Could you check a few things on this drawing? It's one solid part, dimensions in mm from its lowest x, y, z. Coordinates: 2 decimals unless noted, no trailing zeros. Order: outer loops, then holes, each group sorted by start corner. A loop starts at its lowest first (then second) coordinate and runs counter-clockwise, first axis right, second up. Notation, with made-up numbers: (-15, 24.5) - (41, 24.5) arc R19 ccw to (41, 46.5) - close; hole circle Ø3 at (88.5, -37.5). An arc over 180 degrees is marked (long way). Return JSON: item names as keys, results as strings. Group by question number.
1) Imagine slicing it at A-A (z = 0.85). Write out the boundary of the cut face in (x, y), and give its area (3 significant figures).
2) Imagine slicing it at B-B (y = 17.5). Write out the boundary of the cut face in (x, z), and give its area (3 significant figures).
3) If I drill on line 1 along Y through (x, z) = (230, 1.5); line 2 along X through (y, z) = (9, 2.2); line 3 along X through (y, z) = (13, 0.8), over which ranges is the centre line in solid material (lowest first)?
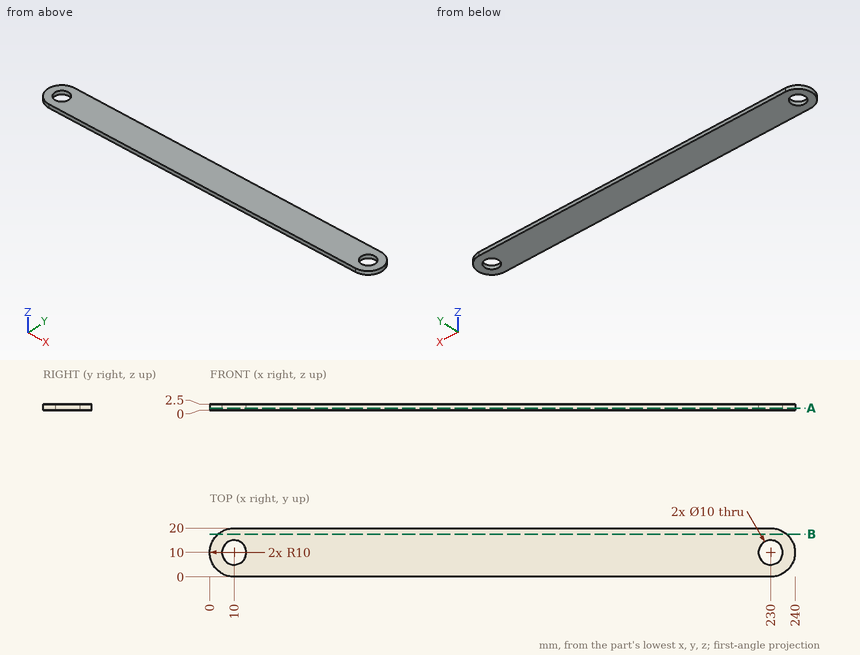
Calculated:
{
 "1": {"outline": "(10, 0) - (230, 0) arc R10 ccw to (230, 20) - (10, 20) arc R10 ccw to start; hole circle Ø10 at (10, 10); hole circle Ø10 at (230, 10)", "area": "4,560 mm2"},
 "2": {"outline": "(3.39, 0) - (236.61, 0) - (236.61, 2.5) - (3.39, 2.5) - close", "area": "583 mm2"},
 "3": {"line 1": "0 to 5, 15 to 20", "line 2": "0.05 to 5.1, 14.9 to 225.1, 234.9 to 239.95", "line 3": "0.46 to 6, 14 to 226, 234 to 239.54"}
}
